Here's how the part is built. I have some questions about the finished solid (model axes, mm). A direction names the side the tool comes from. Coordinates: 2 decimals unless noted, no trailing zeros. Write each loop counter-clockwise with the first axis right and the second up, starting at its lowest first coordinate (ties: lowest second). Pieces come first, ordered by that corner, then holes. Notation, with made-up numbers: (-38.75, 84.5) -> (-25.75, 84.5) arc R30 cw to (-25.75, 108.5) -> close; hole circle Ø10 at (54.5, 38.25). An arc over 180 degrees is marked (long way). Use a Markdown table: item, result. Add a question column.
Item 1: Imagine slicing it at B-B, the plane y = 17. Write out the boundary of the cut face in (x, z), and give its area (3 significant figures).
Item 2: On a 3-axis mill with a long thin cutter (end or side, diameter ignored), from which of +Z, -Z, +X, -X, +Y, -Y can I reach the whole of each face in a straight line? I mean faces 1 (the cylindrical face through (23.797, -33.859, 54.23)), 2 (the flat face through (0, -32, 54)). Say none if no direction works.
Item 3: If I drill on line 1 along X through (y, z) = (10, 55.5); line 2 along Y through (x, z) = (13, 10); line 3 along Y through (x, z) = (23.3, 20), over which ranges is the centre line in solid material (lowest first)? Write a range as from..to.
Item 4: Imagine slicing it at A-A, the plane x = -8.5. Write out the boundary of the cut face in (y, z).
Item 5: If we mould it in two halves opening along Y, with no side actions, what happens to faces 3 (the flat face through (0, 35, 54)), 4 (the flat face through (-22.3, 0.2, 0)), 5 (the flat face through (-22, 0, 54))? For each: pulls with the +Y half, pulls with the -Y half, needs draft (parallel to the pull), parting line crosses it, or undercut.
Item 6: Imagine slicing it at C-C, the plane z = 20. Write out the boundary of the cut face in (x, y).
Item 7: Imagine slicing it at D-D, the plane y = 0. Write out the boundary of the cut face in (x, z), and give its area (3 significant figures).
```python
from build123d import *

# Parameters (mm, degrees)
EXTRUDE_THIN1_DEPTH = 110
SKETCH2_R           = 15.1
CUT_EXTRUDE1_DEPTH  = 126.797456254


with BuildPart() as part:
    # Sketch1 → Extrude-Thin1 (new body)
    with BuildSketch(Plane.XY):
        with BuildLine():
            Line((-25, 31), (-25, -31))
            ThreePointArc((-25, -31), (-23.828427125, -33.828427125), (-21, -35))
            Line((-21, -35), (21, -35))
            ThreePointArc((21, -35), (23.828427125, -33.828427125), (25, -31))
            Line((25, -31), (25, 31))
            ThreePointArc((25, 31), (23.828427125, 33.828427125), (21, 35))
            Line((21, 35), (-21, 35))
            ThreePointArc((-21, 35), (-23.828427125, 33.828427125), (-25, 31))
        make_face()
        with BuildLine():
            Line((-22, 31), (-22, -31))
            ThreePointArc((-22, -31), (-21.707106781, -31.707106781), (-21, -32))
            Line((-21, -32), (21, -32))
            ThreePointArc((21, -32), (21.707106781, -31.707106781), (22, -31))
            Line((22, -31), (22, 31))
            ThreePointArc((22, 31), (21.707106781, 31.707106781), (21, 32))
            Line((21, 32), (-21, 32))
            ThreePointArc((-21, 32), (-21.707106781, 31.707106781), (-22, 31))
        make_face(mode=Mode.SUBTRACT)
    extrude(amount=EXTRUDE_THIN1_DEPTH)

    # Sketch2 → Cut-Extrude1 (cut, through all)
    with BuildSketch(Plane(origin=(25, 0, 0), x_dir=(0, 0, -1), z_dir=(1, 0, 0))):
        with Locations((-20, 0)):
            Circle(SKETCH2_R)
    extrude(amount=-CUT_EXTRUDE1_DEPTH, mode=Mode.SUBTRACT)


solid = part.part
```
Ans:
| question | item | result |
|---|---|---|
| 1 | outline | (-25, 0) -> (-22, 0) -> (-22, 110) -> (-25, 110) -> close; (22, 0) -> (25, 0) -> (25, 110) -> (22, 110) -> close |
| 1 | area | 660 mm^2 |
| 2 | face 1 | +Z, -Z, +X, -Y |
| 2 | face 2 | +Z, -Z |
| 3 | line 1 | x = -25..-22, 22..25 |
| 3 | line 2 | y = -35..-32, 32..35 |
| 3 | line 3 | y = -34.27..-15.1, 15.1..34.27 |
| 4 | outline | (-35, 0) -> (-32, 0) -> (-32, 110) -> (-35, 110) -> close; (32, 0) -> (35, 0) -> (35, 110) -> (32, 110) -> close |
| 5 | face 3 | pulls with the +Y half |
| 5 | face 4 | needs draft |
| 5 | face 5 | undercut |
| 6 | outline | (-25, -31) arc R4 ccw to (-21, -35) -> (21, -35) arc R4 ccw to (25, -31) -> (25, -15.1) -> (22, -15.1) -> (22, -31) arc R1 cw to (21, -32) -> (-21, -32) arc R1 cw to (-22, -31) -> (-22, -15.1) -> (-25, -15.1) -> close; (-25, 15.1) -> (-22, 15.1) -> (-22, 31) arc R1 cw to (-21, 32) -> (21, 32) arc R1 cw to (22, 31) -> (22, 15.1) -> (25, 15.1) -> (25, 31) arc R4 ccw to (21, 35) -> (-21, 35) arc R4 ccw to (-25, 31) -> close |
| 7 | outline | (-25, 0) -> (-22, 0) -> (-22, 4.9) -> (-25, 4.9) -> close; (-25, 35.1) -> (-22, 35.1) -> (-22, 110) -> (-25, 110) -> close; (22, 0) -> (25, 0) -> (25, 4.9) -> (22, 4.9) -> close; (22, 35.1) -> (25, 35.1) -> (25, 110) -> (22, 110) -> close |
| 7 | area | 479 mm^2 |
